The model under review builds one solid part; all positions refer to its coordinate system, in mm. Round coordinates to 2 decimals unless told otherwise and drop trailing zeros. Write each loop counter-clockwise with the first axis right and the second up, starting at its lowest first coordinate (ties: lowest second). Pieces come first, ordered by that corner, then holes. Notation, with made-up numbers: (65, 7) - (115, 7) arc R30 ccw to (115, 31) - close; hole circle Ø2 at (69.25, -28.5). An arc over 180 degrees is marked (long way). Return JSON: item names as keys, results as strings.
from build123d import *

# Parameters (mm, degrees)
HEX_BODY_DEPTH          = 3
HEX_CORNER_FILLETS_R1_R = 1
BORE_SKETCH_R           = 4
BORE_8_DEPTH            = 3


with BuildPart() as part:
    # Hex Profile Sketch → Hex Body (new body)
    with BuildSketch(Plane.XY):
        Polygon((3.5, -6.062177826), (7, 0), (3.5, 6.062177826), (-3.5, 6.062177826), (-7, 0), (-3.5, -6.062177826), align=None)
    extrude(amount=HEX_BODY_DEPTH)

    # Hex Corner Fillets R1
    hex_corner_fillets_r1_edges = [part.edges().sort_by_distance(p)[0] for p in [
        (-3.5, -6.062177826, 1.5),
        (-7, 0, 1.5),
        (-3.5, 6.062177826, 1.5),
        (3.5, 6.062177826, 1.5),
        (7, 0, 1.5),
        (3.5, -6.062177826, 1.5),
    ]]
    fillet(hex_corner_fillets_r1_edges, radius=HEX_CORNER_FILLETS_R1_R)

    # Bore Sketch → Bore Ø8 (cut)
    with BuildSketch(Plane.XY.offset(3)):
        Circle(BORE_SKETCH_R)
    extrude(amount=-BORE_8_DEPTH, mode=Mode.SUBTRACT)


solid = part.part
(1) Add section A-A (z = 0.45). Write out the cut boundary in (x, y), plus the area to 3 significant figures.
Filled in:
{"outline": "(-6.71, -0.5) - (-3.79, -5.56) arc R1 ccw to (-2.92, -6.06) - (2.92, -6.06) arc R1 ccw to (3.79, -5.56) - (6.71, -0.5) arc R1 ccw to (6.71, 0.5) - (3.79, 5.56) arc R1 ccw to (2.92, 6.06) - (-2.92, 6.06) arc R1 ccw to (-3.79, 5.56) - (-6.71, 0.5) arc R1 ccw to start; hole circle Ø8 at (0, 0)", "area": "76.7 mm2"}
(2) Add section B-B (y = 0). Write out the cut boundary in (x, z), plus the area to 3 significant figures.
Filled in:
{"outline": "(-6.85, 0) - (-4, 0) - (-4, 3) - (-6.85, 3) - close; (4, 0) - (6.85, 0) - (6.85, 3) - (4, 3) - close", "area": "17.1 mm2"}
(3) Mouldability with a two-part tool opening along X and no side actions: class faces 1 (the cylindrical face through (-0.867, -3.905, 1.521)), 2 (the flat face through (-5.23, 3.067, 1.479)), 3 (the flat face through (5.27, 3, 1.48)), 4 (the flat face through (0, 6.062, 1)) as released by +X, released by -X, zero draft, split by the parting line, or undercut.
Filled in:
{"face 1": "undercut", "face 2": "released by -X", "face 3": "released by +X", "face 4": "zero draft"}
(4) Clearance check with a flat-ended pin moving along its axis: pin 1 Ø1 at (x, z) = (3.5, 2) entering from +Y. State where the tip first meets the part, or that it passes through.
Filled in:
{"pin 1": "stops at y = 6.06"}
(5) Add section C-C (x = 0.75). Write out the cut boundary in (y, z), plus the area to 3 significant figures.
Filled in:
{"outline": "(-6.06, 0) - (-3.93, 0) - (-3.93, 3) - (-6.06, 3) - close; (3.93, 0) - (6.06, 0) - (6.06, 3) - (3.93, 3) - close", "area": "12.8 mm2"}
(6) Add section D-D (y = -4.25). Write out the cut boundary in (x, z), plus the area to 3 significant figures.
Filled in:
{"outline": "(-4.55, 0) - (4.55, 0) - (4.55, 3) - (-4.55, 3) - close", "area": "27.3 mm2"}
(7) Wall thickness on line 1 (Y direction, x = 0, z = 1.1); line 2 (X direction, y = -2.5, z = 2.3); line 3 (X direction, y = 1.25, z = 1.35): over which ranges is each line inside the solid? List them lowest first.
Filled in:
{"line 1": "y = -6.06 to -4, 4 to 6.06", "line 2": "x = -5.56 to -3.12, 3.12 to 5.56", "line 3": "x = -6.28 to -3.8, 3.8 to 6.28"}
